Part model, mm, in its own coordinate system. Face numbers are marked on the shaded views. A direction names the side the tool comes from. Give positions to 0.01 mm unless a question says otherwise; leave off trailing zeros. Loops run counter-clockwise (first coordinate to the right, second up) from the corner with the lowest first, then second, coordinate; pieces in that order, holes last. Notation, with made-up numbers: M 14.5,67.5 L 69.5,67.5 A17 ccw 69.5,79.5 Z; hole C 75,11.25 d11. An arc over 180 degrees is marked long. Answer in a Markdown table with one row per item.
from build123d import *

# Parameters (mm, degrees)
BASE_PLATE_DEPTH         = 30
CENTER_BORE_PROFILE_R    = 20
CENTER_BORE_DEPTH        = 30
SIDE_HOLES_PROFILE_R     = 10
SIDE_HOLES_2X_28_DEPTH   = 30
LUG_1_DEPTH              = 50
LUG_1_TAPER_CUT_DEPTH    = 35
LUG_1_PIN_HOLE_PROFILE_R = 5
LUG_1_PIN_HOLE_DEPTH     = 15
LUG_START                = -50
LUG_2_DEPTH              = 50
LUG_START_2              = -35
LUG_2_TAPER_CUT_DEPTH    = 35
LUG_START_3              = -15
LUG_2_PIN_HOLE_PROFILE_R = 5
LUG_2_PIN_HOLE_DEPTH     = 15


with BuildPart() as part:
    # Base Plate Profile → Base Plate (new body)
    with BuildSketch(Plane.XY):
        with BuildLine():
            Line((0, 0), (140, 0))
            Line((140, 0), (140, 56))
            Line((140, 56), (125, 56))
            ThreePointArc((125, 56), (114.393398282, 60.393398282), (110, 71))
            Line((110, 71), (110, 76))
            ThreePointArc((110, 76), (70, 116), (30, 76))
            Line((30, 76), (30, 70))
            ThreePointArc((30, 70), (25.606601718, 59.393398282), (15, 55))
            Line((15, 55), (0, 55))
            Line((0, 55), (0, 0))
        make_face()
    extrude(amount=BASE_PLATE_DEPTH)

    # Center Bore Profile → Center Bore (cut)
    with BuildSketch(Plane.XY.offset(30)):
        with Locations((70, 76)):
            Circle(CENTER_BORE_PROFILE_R)
    extrude(amount=-CENTER_BORE_DEPTH, mode=Mode.SUBTRACT)

    # Side Holes Profile → Side Holes 2xØ28 (cut)
    with BuildSketch(Plane.XY.offset(30)):
        with Locations((15.451626978, 28)):
            Circle(SIDE_HOLES_PROFILE_R)
        with Locations((123.451626978, 28)):
            Circle(SIDE_HOLES_PROFILE_R)
    extrude(amount=-SIDE_HOLES_2X_28_DEPTH, mode=Mode.SUBTRACT)

    # Lug 1 Profile → Lug 1 (add)
    with BuildSketch(Plane.ZY):
        with BuildLine():
            Line((30, 0), (30, 45))
            Line((30, 45), (66, 18))
            ThreePointArc((66, 18), (69.486832981, 6.83772234), (60, 0))
            Line((60, 0), (30, 0))
        make_face()
    extrude(amount=-LUG_1_DEPTH)

    # Lug 1 Taper Profile → Lug 1 Taper Cut (cut)
    with BuildSketch(Plane.ZY):
        with BuildLine():
            Line((30, 45), (30, 0))
            Line((30, 0), (60, 0))
            ThreePointArc((60, 0), (69.486832981, 6.83772234), (66, 18))
            Line((66, 18), (30, 45))
        make_face()
    extrude(amount=-LUG_1_TAPER_CUT_DEPTH, mode=Mode.SUBTRACT)

    # Lug 1 Pin Hole Profile → Lug 1 Pin Hole (cut)
    with BuildSketch(Plane.ZY.offset(-35)):
        with Locations((60, 10)):
            Circle(LUG_1_PIN_HOLE_PROFILE_R)
    extrude(amount=-LUG_1_PIN_HOLE_DEPTH, mode=Mode.SUBTRACT)

    # Lug 2 Profile → Lug 2 (add)
    with BuildSketch(Plane(origin=(140, 0, 0), x_dir=(0, 0, -1), z_dir=(1, 0, 0)).offset(LUG_START)):
        with BuildLine():
            Line((-30, 0), (-30, 45))
            Line((-30, 45), (-66, 18))
            ThreePointArc((-66, 18), (-69.486832981, 6.83772234), (-60, 0))
            Line((-60, 0), (-30, 0))
        make_face()
    extrude(amount=LUG_2_DEPTH)

    # Lug 2 Taper Profile → Lug 2 Taper Cut (cut)
    with BuildSketch(Plane(origin=(140, 0, 0), x_dir=(0, 0, -1), z_dir=(1, 0, 0)).offset(LUG_START_2)):
        with BuildLine():
            Line((-30, 45), (-66, 18))
            ThreePointArc((-66, 18), (-69.486832981, 6.83772234), (-60, 0))
            Line((-60, 0), (-30, 0))
            Line((-30, 0), (-30, 45))
        make_face()
    extrude(amount=LUG_2_TAPER_CUT_DEPTH, mode=Mode.SUBTRACT)

    # Lug 2 Pin Hole Profile → Lug 2 Pin Hole (cut)
    with BuildSketch(Plane(origin=(105, 0, 0), x_dir=(0, 0, -1), z_dir=(1, 0, 0)).offset(LUG_START_3)):
        with Locations(Location((-60, 10, 0), (0, 0, 180))):
            Circle(LUG_2_PIN_HOLE_PROFILE_R)
    extrude(amount=LUG_2_PIN_HOLE_DEPTH, mode=Mode.SUBTRACT)


solid = part.part
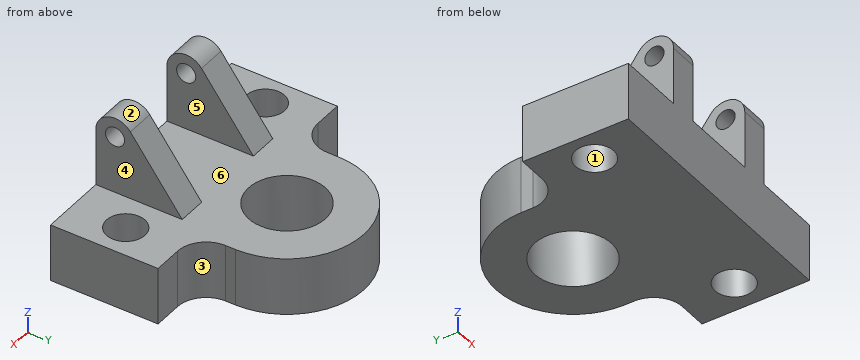
(1) Pull direction X, two halves, no side cores. Call the marked faces 1, 2 and 3: +X half, -X half, draft (parallel to the pull), parting line (faces both ways), or undercut.
Recorded:
| item | result |
|---|---|
| face 1 | undercut |
| face 2 | draft |
| face 3 | +X half |
(2) Saw through at B-B (z = 32). Write the cut outline in (x, y).
Recorded:
| item | result |
|---|---|
| outline | M 35,0 L 50,0 L 50,43.5 L 35,43.5 Z; M 90,0 L 105,0 L 105,43.5 L 90,43.5 Z |
(3) Which spindle directions (+Z, -Z, +X, -X, +Y, -Y) get a long thin tool onto all of the face, cutting with end or side? Do the marked faces 4, 5 and 6. Say none if no direction does.
Recorded:
| item | result |
|---|---|
| face 4 | +Z, +X, +Y, -Y |
| face 5 | +Z, +Y, -Y |
| face 6 | +Z, +Y |
(4) Pin check, flat tips, straight feed: pin 1 Ø20 at (y, z) = (32.5, 45) entering from +X; pin 2 Ø1.5 at (y, z) = (73, 10.5) entering from +X; pin 3 Ø4.5 at (x, z) = (133.5, 19) entering from +Y; pin 4 Ø4 at (x, z) = (63, 32.5) entering from -Y. Stop position of each tip, or through.
Recorded:
| item | result |
|---|---|
| pin 1 | stops at x = 105 |
| pin 2 | stops at x = 110 |
| pin 3 | stops at y = 56 |
| pin 4 | passes through |
(5) Saw through at C-C (x = 70). Write the cut outline in (y, z).
Recorded:
| item | result |
|---|---|
| outline | M 0,0 L 56,0 L 56,30 L 0,30 Z; M 96,0 L 116,0 L 116,30 L 96,30 Z |
(6) Saw through at A-A (y = 10). Write the cut outline in (x, z).
Recorded:
| item | result |
|---|---|
| outline | M 0,0 L 140,0 L 140,30 L 105,30 L 105,55 L 90,55 L 90,30 L 50,30 L 50,55 L 35,55 L 35,30 L 0,30 Z; M 35,65 L 50,65 L 50,70 L 35,70 Z; M 90,65 L 105,65 L 105,70 L 90,70 Z |
(7) Saw through at D-D (z = 14). Write the cut outline in (x, y), plus the area to 3 significant figures.
Recorded:
| item | result |
|---|---|
| outline | M 0,0 L 140,0 L 140,56 L 125,56 A15 cw 110,71 L 110,76 A40 ccw 30,76 L 30,70 A15 cw 15,55 L 0,55 Z; hole C 15.45,28 d20; hole C 70,76 d40; hole C 123.45,28 d20 |
| area | 10,100 mm^2 |
(8) Drill centre lines: line 1 along Z through (x, y) = (101.75, 10); line 2 along X through (y, z) = (34.5, 11); line 3 along Y through (x, z) = (70, 11). Where is each one in solid material? Low to high.
Recorded:
| item | result |
|---|---|
| line 1 | z = 0 to 55, 65 to 70 |
| line 2 | x = 0 to 7.85, 23.05 to 115.85, 131.05 to 140 |
| line 3 | y = 0 to 56, 96 to 116 |
